```python
from build123d import *

# Parameters (mm, degrees)
SKETCH_1_W      = 120
SKETCH_1_H      = 90
EXTRUDE_1_DEPTH = 45
SKETCH_2_R      = 8
EXTRUDE_2_DEPTH = 80


with BuildPart() as part:
    # 草图1 → 凸台-拉伸1 (new, symmetric)
    with BuildSketch(Plane.XY):
        Rectangle(SKETCH_1_W, SKETCH_1_H)
    extrude(amount=EXTRUDE_1_DEPTH, both=True)

    # 草图2 → 凸台-拉伸2 (add, symmetric)
    with BuildSketch(Plane.XY):
        Circle(SKETCH_2_R)
    extrude(amount=EXTRUDE_2_DEPTH, both=True)


solid = part.part
```
Model file for the job. Use its own axes, mm. A direction names the side the tool comes from. Coordinates: 2 decimals unless noted, no trailing zeros. Loops run counter-clockwise (first coordinate to the right, second up) from the corner with the lowest first, then second, coordinate; pieces in that order, holes last. Notation, with made-up numbers: (-7.75, 72.25) -> (45.25, 72.25) arc R13 ccw to (45.25, 92.25) -> close; hole circle Ø2 at (40, 34.5). An arc over 180 degrees is marked (long way). Answer as a JSON object with one key per item and string values.
Q1. Probe probe 1 along Z at (x, y) = (37, -36); probe 2 along X at (y, z) = (-2, -70). List the from-to ranges inside material, lowest first.
Report:
{"probe 1": "z = -45 to 45", "probe 2": "x = -7.75 to 7.75"}
Q2. Flat gauge pins, fed straight in: P1, Ø12, axis at x = 33, y = -18, coming from the +Z side; P2, Ø12, axis at x = -29.5, z = 55, coming from the +Y side. Where does each tip first touch, or does it go through?
Report:
{"P1": "stops at z = 45", "P2": "passes through"}
Q3. Pull direction Z, two halves, no side cores. Call faces 3 (the flat face through (0, 0, -80)), 4 (the cylindrical face through (-1.73, -7.81, 62.74)), 5 (the flat face through (0, 0, 80)): released by +Z, released by -Z, zero draft, split by the parting line, or undercut.
Report:
{"face 3": "released by -Z", "face 4": "zero draft", "face 5": "released by +Z"}
Q4. Cut at D-D (y = 34). List the corners of the cut face in (x, z), and give its area (3 significant figures).
Report:
{"outline": "(-60, -45) -> (60, -45) -> (60, 45) -> (-60, 45) -> close", "area": "10,800 mm2"}
Q5. Cut at A-A (y = 0). List the corners of the cut face in (x, z).
Report:
{"outline": "(-60, -45) -> (-8, -45) -> (-8, -80) -> (8, -80) -> (8, -45) -> (60, -45) -> (60, 45) -> (8, 45) -> (8, 80) -> (-8, 80) -> (-8, 45) -> (-60, 45) -> close"}
Q6. Cut at B-B (x = 0). List the corners of the cut face in (y, z), and give its area (3 significant figures).
Report:
{"outline": "(-45, -45) -> (-8, -45) -> (-8, -80) -> (8, -80) -> (8, -45) -> (45, -45) -> (45, 45) -> (8, 45) -> (8, 80) -> (-8, 80) -> (-8, 45) -> (-45, 45) -> close", "area": "9,220 mm2"}
Q7. 3-axis set-ups, long thin cutter, end or side, ignore diameter. For faces 1 (the cylindrical face through (-1.73, -7.81, -62.26)), 2 (the flat face through (-60, -1, 1)): which of +Z, -Z, +X, -X, +Y, -Y reach the whole face in a straight line?
Report:
{"face 1": "-Z", "face 2": "+Z, -Z, -X, +Y, -Y"}
Q8. Cut at C-C (z = -65.5). List the corners of the cut face in (x, y).
Report:
{"outline": "circle Ø16 at (0, 0)"}
